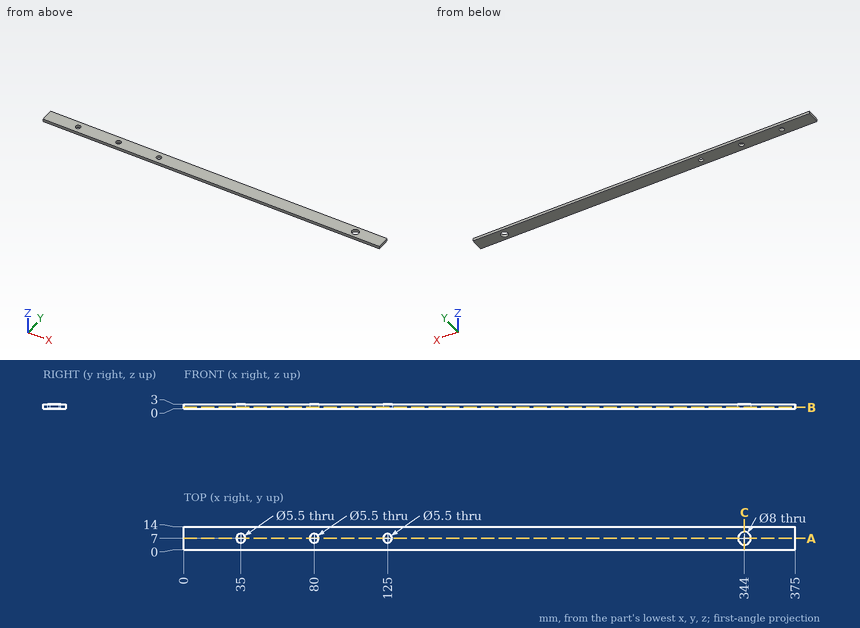
Source: three-view drawing plus pictorial views. Frame: mm from the lowest corner of the part. Give positions to 0.01 mm unless a question says otherwise; leave off trailing zeros. Order: outer loops, then holes, each group sorted by start corner. A loop starts at its lowest first (then second) coordinate and runs counter-clockwise, first axis right, second up. Notation, with made-up numbers: (11, 83) - (66, 83) arc R34 cw to (66, 122) - close; hole circle Ø6 at (40.5, -3.5). An arc over 180 degrees is marked (long way). Answer as a JSON object with one key per item and string values. Group by question number.
Q1. Line query: probe 1 along Y at (x, z) = (125, 2.15); probe 2 along X at (y, z) = (9.5, 1.4); probe 3 along X at (y, z) = (8.75, 2.5). Output: solid intervals per line, ascending.
Q2. First-contact query: pin 1 Ø4.5 at (x, y) = (35, 7) entering from +Z. Flat tip, straight axial feed; report the tip coordinate or a pass-through.
Q3. Cut plane C-C, the plane x = 344. Output: boundary loops of the cut face in (y, z).
Q4. Cut plane B-B, the plane z = 1. Output: boundary loops of the cut face in (x, y).
Q5. Cut plane A-A, the plane y = 7. Output: boundary loops of the cut face in (x, z).
Results:
{
 "1": {"probe 1": "0 to 4.25, 9.75 to 14", "probe 2": "0 to 33.85, 36.15 to 78.85, 81.15 to 123.85, 126.15 to 340.88, 347.12 to 375", "probe 3": "0 to 32.88, 37.12 to 77.88, 82.12 to 122.88, 127.12 to 340.4, 347.6 to 375"},
 "2": {"pin 1": "through"},
 "3": {"outline": "(0, 0) - (3, 0) - (3, 3) - (0, 3) - close; (11, 0) - (14, 0) - (14, 3) - (11, 3) - close"},
 "4": {"outline": "(0, 0) - (375, 0) - (375, 14) - (0, 14) - close; hole circle Ø5.5 at (35, 7); hole circle Ø5.5 at (80, 7); hole circle Ø5.5 at (125, 7); hole circle Ø8 at (344, 7)"},
 "5": {"outline": "(0, 0) - (32.25, 0) - (32.25, 3) - (0, 3) - close; (37.75, 0) - (77.25, 0) - (77.25, 3) - (37.75, 3) - close; (82.75, 0) - (122.25, 0) - (122.25, 3) - (82.75, 3) - close; (127.75, 0) - (340, 0) - (340, 3) - (127.75, 3) - close; (348, 0) - (375, 0) - (375, 3) - (348, 3) - close"}
}
